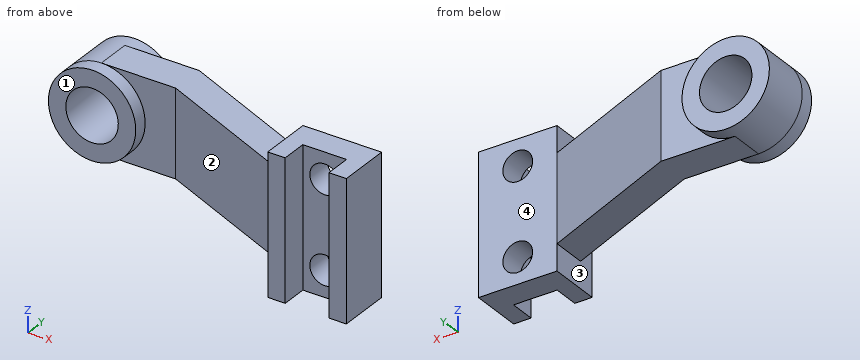
from build123d import *

# Parameters (mm, degrees)
ARM_BODY_DEPTH            = 80
END_BLOCK_DEPTH           = 60
END_BLOCK_SLOT_CUT_DEPTH  = 15
END_BLOCK_PAD_5MM_DEPTH   = 5
MOUNTING_HOLES_SKETCH_R   = 8.5
MOUNTING_HOLES_2X_DEPTH   = 15
ARM_RELIEF_CUT_DEPTH      = 55
ARM_WEB_SKETCH_W          = 42.5
ARM_WEB_SKETCH_H          = 20
ARM_WEB_DEPTH             = 50
HUB_FLANGE_LOWER_SKETCH_R = 25
HUB_FLANGE_LOWER_50_DEPTH = 8
HUB_START                 = 20
HUB_BODY_DEPTH            = 20
HUB_START_2               = 8
HUB_FLANGE_UPPER_SKETCH_R = 25
HUB_FLANGE_UPPER_50_DEPTH = 8
HUB_BORE_SKETCH_R         = 15
HUB_BORE_30_DEPTH         = 40


with BuildPart() as part:
    # Arm Profile Sketch → Arm Body (new body)
    with BuildSketch(Plane.XY):
        Polygon((0, 0), (10, 0), (10, 15), (35, 15), (35, 0), (45, 0), (45, 30), (0, 30), align=None)
    extrude(amount=ARM_BODY_DEPTH)

    # End Block Sketch → End Block (add)
    with BuildSketch(Plane.XY.offset(80)):
        Polygon((-102.5, 75), (-102.5, 55), (0, 10), (0, 30), align=None)
    extrude(amount=-END_BLOCK_DEPTH)

    # End Block Slot Sketch → End Block Slot Cut (cut)
    with BuildSketch(Plane.XY.offset(80)):
        Polygon((-102.5, 75), (0, 30), (0, 10), (-102.5, 55), align=None)
    extrude(amount=-END_BLOCK_SLOT_CUT_DEPTH, mode=Mode.SUBTRACT)

    # End Block Pad Sketch → End Block Pad 5mm (add)
    with BuildSketch(Plane(origin=(0, 0, 20), x_dir=(-1, 0, 0), z_dir=(0, 0, -1))):
        Polygon((0, 30), (102.5, 75), (102.5, 55), (0, 10), align=None)
    extrude(amount=END_BLOCK_PAD_5MM_DEPTH)

    # Mounting Holes Sketch → Mounting Holes 2x (cut)
    with BuildSketch(Plane(origin=(0, 30, 0), x_dir=(1, 0, 0), z_dir=(0, 1, 0))):
        with Locations(Location((22.5, -15, 0), (0, 0, 270))):
            Circle(MOUNTING_HOLES_SKETCH_R)
        with Locations(Location((22.5, -65, 0), (0, 0, 270))):
            Circle(MOUNTING_HOLES_SKETCH_R)
    extrude(amount=-MOUNTING_HOLES_2X_DEPTH, mode=Mode.SUBTRACT)

    # Arm Relief Cut Sketch → Arm Relief Cut (cut)
    with BuildSketch(Plane.XY.offset(65)):
        Polygon((-102.5, 75), (-84.187119396, 66.960198759), (-84.187119396, 46.960198759), (-102.5, 55), align=None)
    extrude(amount=-ARM_RELIEF_CUT_DEPTH, mode=Mode.SUBTRACT)

    # Arm Web Sketch → Arm Web (add)
    with BuildSketch(Plane.XY.offset(65)):
        with Locations((-105.437119396, 56.960198759)):
            Rectangle(ARM_WEB_SKETCH_W, ARM_WEB_SKETCH_H)
    extrude(amount=-ARM_WEB_DEPTH)

    # Hub Flange Lower Sketch → Hub Flange Lower Ø50 (add)
    with BuildSketch(Plane(origin=(0, 66.960198759, 0), x_dir=(1, 0, 0), z_dir=(0, 1, 0))):
        with Locations(Location((-126.687119396, -40, 0), (0, 0, 270))):
            Circle(HUB_FLANGE_LOWER_SKETCH_R)
    extrude(amount=HUB_FLANGE_LOWER_50_DEPTH)

    # Hub Body Sketch → Hub Body (add)
    with BuildSketch(Plane.XZ.offset(-66.960198759).offset(HUB_START)):
        with BuildLine():
            Line((-126.687119396, 65), (-126.687119396, 15))
            ThreePointArc((-126.687119396, 15), (-151.687119396, 40), (-126.687119396, 65))
        make_face()
    extrude(amount=-HUB_BODY_DEPTH)

    # Hub Flange Upper Sketch → Hub Flange Upper Ø50 (add)
    with BuildSketch(Plane.XZ.offset(-46.960198759).offset(HUB_START_2)):
        with Locations(Location((-126.687119396, 40, 0), (0, 0, 270))):
            Circle(HUB_FLANGE_UPPER_SKETCH_R)
    extrude(amount=-HUB_FLANGE_UPPER_50_DEPTH)

    # Hub Bore Sketch → Hub Bore Ø30 (cut)
    with BuildSketch(Plane(origin=(0, 74.960198759, 0), x_dir=(1, 0, 0), z_dir=(0, 1, 0))):
        with Locations(Location((-126.687119396, -40, 0), (0, 0, 270))):
            Circle(HUB_BORE_SKETCH_R)
    extrude(amount=-HUB_BORE_30_DEPTH, mode=Mode.SUBTRACT)


solid = part.part
Design review of the part built by this model. Coordinates are the model's own, in mm. Face numbers are marked on the shaded views. A direction names the side the tool comes from. Coordinates: 2 decimals unless noted, no trailing zeros. Write each loop counter-clockwise with the first axis right and the second up, starting at its lowest first coordinate (ties: lowest second). Pieces come first, ordered by that corner, then holes. Notation, with made-up numbers: (83, 41.5) -> (99, 41.5) arc R13 ccw to (99, 50.5) -> close; hole circle Ø2 at (85.5, 69.25). An arc over 180 degrees is marked (long way). Write each question's results on one line, items separated by ' | '. Start each with the question number.
(1) For line 1 along Z through (x, y) = (22, 20); line 2 along X through (y, z) = (6, 75); line 3 along X through (y, z) = (39, 48), list the stretches that pass through material, from the lowest coordinate up. Write a range as from..to.
(2) Take a section at C-C on y = 24.5. Write out the cut boundary in (x, z), and give its area (3 significant figures).
(3) Take a section at D-D on x = -114. Write out the cut boundary in (y, z).
(4) Tool access review of the marked faces 1, 2, 3 and 4: name each direction out of +Z, -Z, +X, -X, +Y, -Y from which nothing blocks a thin tool from reaching the whole face with its end or side.
(5) Clearance check with flat-ended pins moving along their axes: P1, Ø10, axis at x = -37.5, y = 42, coming from the +Z side; P2, Ø19.5, axis at x = 22.5, z = 15, coming from the -Y side; P3, Ø15, axis at x = -120.5, z = 28, coming from the -Y side; P4, Ø10, axis at x = -126.5, z = 51.5, coming from the +Y side. State where each tip first meets the part, or that it passes through.
(6) Take a section at A-A on z = 40. Write out the cut boundary in (x, y).
(7) Take a section at B-B on x = 22.5. Write out the cut boundary in (y, z).
Results found:
1) line 1: z = 0..6.51, 23.49..56.51, 73.49..80 | line 2: x = 0..10, 35..45 | line 3: x = -150.37..-139.38, -114..-103, -66.06..-20.5
2) outline: (-33.03, 15) -> (0, 15) -> (0, 0) -> (45, 0) -> (45, 80) -> (0, 80) -> (0, 65) -> (-33.03, 65) -> close; hole circle Ø17 at (22.5, 15); hole circle Ø17 at (22.5, 65) | area: 4,800 mm2
3) outline: (38.96, 18.46) -> (46.96, 18.46) -> (46.96, 15) -> (66.96, 15) -> (66.96, 18.46) -> (74.96, 18.46) -> (74.96, 32) -> (38.96, 32) -> close; (38.96, 48) -> (74.96, 48) -> (74.96, 61.54) -> (66.96, 61.54) -> (66.96, 65) -> (46.96, 65) -> (46.96, 61.54) -> (38.96, 61.54) -> close
4) face 1: +Z, -Z, -X, -Y | face 2: +Z, -Z, -Y | face 3: -X, -Y | face 4: +Z, -Z, +X, +Y
5) P1: stops at z = 65 | P2: stops at y = 15 | P3: stops at y = 38.96 | P4: stops at y = 74.96
6) outline: (-151.69, 38.96) -> (-141.69, 38.96) -> (-141.69, 74.96) -> (-151.69, 74.96) -> close; (-111.69, 38.96) -> (-101.69, 38.96) -> (-101.69, 46.96) -> (-84.19, 46.96) -> (0, 10) -> (0, 0) -> (10, 0) -> (10, 15) -> (35, 15) -> (35, 0) -> (45, 0) -> (45, 30) -> (0, 30) -> (-84.19, 66.96) -> (-101.69, 66.96) -> (-101.69, 74.96) -> (-111.69, 74.96) -> close
7) outline: (15, 0) -> (30, 0) -> (30, 6.5) -> (15, 6.5) -> close; (15, 23.5) -> (30, 23.5) -> (30, 56.5) -> (15, 56.5) -> close; (15, 73.5) -> (30, 73.5) -> (30, 80) -> (15, 80) -> close
